from build123d import *

# Parameters (mm, degrees)
SKETCH_1_W              = 50
SKETCH_1_H              = 55
EXTRUDE_1_DEPTH         = 30
CHAMFER_1_SIZE          = 20
HOLE_WIZARD_M10_1_D     = 8.5
HOLE_WIZARD_M10_1_DEPTH = 24.5
HOLE_WIZARD_M10_1_TIP   = 2.553657631
SKETCH_5_R              = 6.25
CUT_EXTRUDE_1_DEPTH     = 30


with BuildPart() as part:
    # 草图1 → 凸台-拉伸1 (new body)
    with BuildSketch(Plane.XY):
        Rectangle(SKETCH_1_W, SKETCH_1_H)
    extrude(amount=EXTRUDE_1_DEPTH)

    # 倒角1
    chamfer_1_edges = [part.edges().sort_by_distance(p)[0] for p in [
        (-25, 27.5, 15),
        (25, 27.5, 15),
    ]]
    chamfer(chamfer_1_edges, length=CHAMFER_1_SIZE)

    # M10 螺纹孔1
    with Locations(Plane(origin=(0, -27.5, 0), x_dir=(-1, 0, 0), z_dir=(0, -1, 0))):
        with Locations((15, -15), (-15, -15)):
            Hole(HOLE_WIZARD_M10_1_D / 2, depth=HOLE_WIZARD_M10_1_DEPTH)
            with Locations((0, 0, -(HOLE_WIZARD_M10_1_DEPTH + HOLE_WIZARD_M10_1_TIP / 2))):  # 118° drill point
                Cone(0, HOLE_WIZARD_M10_1_D / 2, HOLE_WIZARD_M10_1_TIP, mode=Mode.SUBTRACT)

    # 草图5 → 切除-拉伸1 (cut)
    with BuildSketch(Plane.XY.offset(30)):
        with Locations((0, 10.2)):
            Circle(SKETCH_5_R)
    extrude(amount=-CUT_EXTRUDE_1_DEPTH, mode=Mode.SUBTRACT)


solid = part.part
CAD build for the part. Positions are in the model's coordinates, mm. A direction names the side the tool comes from. Coordinates: 2 decimals unless noted, no trailing zeros. Loops run counter-clockwise (first coordinate to the right, second up) from the corner with the lowest first, then second, coordinate; pieces in that order, holes last. Notation, with made-up numbers: (6, -38) - (21, -38) arc R20 ccw to (21, -33) - close; hole circle Ø7 at (-30.75, 58). An arc over 180 degrees is marked (long way). Write item = value, one per line. Start each with the question number.
Q1. Flat gauge pins, fed straight in: pin 1 Ø11 at (x, z) = (15, 15) entering from +Y; pin 2 Ø8 at (x, z) = (13, 15) entering from +Y; pin 3 Ø10 at (x, z) = (-15, 15) entering from +Y. Where does each tip first touch, or does it go through?
Q2. Cut at B-B, the plane z = 22. List the corners of the cut face in (x, y).
Q3. Cut at C-C, the plane x = 0. List the corners of the cut face in (y, z).
Q4. Which spindle directions (+Z, -Z, +X, -X, +Y, -Y) get a long thin tool onto all of the face, cutting with end or side? Do faces 5 (the flat face through (0, -6, 30)), 6 (the cylindrical face through (14.08, -15.08, 19.15)). Say none if no direction does.
Q5. Pull direction X, two halves, no side cores. Call faces 1 (the cylindrical face through (-13.04, -15.08, 18.77)), 2 (the flat face through (-14.9, 17.6, 14.8)), 3 (the cylindrical face through (3.36, 15.47, 15.21)), 4 (the flat face through (0, -27.5, 15)): pulls with the +X half, pulls with the -X half, needs draft (parallel to the pull), parting line crosses it, or undercut.
Q6. Drill centre lines: L1, parallel to Z at x = 15, y = -13.5; L2, parallel to Y at x = -7.5, z = 22; L3, parallel to X at y = 7.5, z = 29. Where is each one in solid material? Low to high.
Q7. Cut at D-D, the plane y = -12. List the corners of the cut face in (x, z).
Q8. Cut at A-A, the plane y = 10.2. List the corners of the cut face in (x, z).
Computed:
q1.pin_1 = 23
q1.pin_2 = 23.5
q1.pin_3 = 22.5
q2.outline = (-25, -27.5) - (25, -27.5) - (25, 7.5) - (5, 27.5) - (-5, 27.5) - (-25, 7.5) - close; hole circle Ø12.5 at (0, 10.2)
q3.outline = (-27.5, 0) - (3.95, 0) - (3.95, 30) - (-27.5, 30) - close; (16.45, 0) - (27.5, 0) - (27.5, 30) - (16.45, 30) - close
q4.face_5 = +Z, +X, -X, +Y, -Y
q4.face_6 = -Y
q5.face_1 = undercut
q5.face_2 = pulls with the -X half
q5.face_3 = undercut
q5.face_4 = needs draft
q6.L1 = 0 to 10.75, 19.25 to 30
q6.L2 = -27.5 to 25
q6.L3 = -25 to -5.64, 5.64 to 25
q7.outline = (-25, 0) - (25, 0) - (25, 30) - (-25, 30) - close; hole circle Ø8.5 at (-15, 15); hole circle Ø8.5 at (15, 15)
q8.outline = (-22.3, 0) - (-6.25, 0) - (-6.25, 30) - (-22.3, 30) - close; (6.25, 0) - (22.3, 0) - (22.3, 30) - (6.25, 30) - close
